Source: CAD feature listing. Evaluate the final solid. Frame: model axes, mm. Face numbers are marked on the shaded views. Give positions to 0.01 mm unless a question says otherwise; leave off trailing zeros. Loops run counter-clockwise (first coordinate to the right, second up) from the corner with the lowest first, then second, coordinate; pieces in that order, holes last. Notation, with made-up numbers: M -28,-6 L -12,-6 A18 cw -12,27 Z; hole C 35,62.25 d2. An arc over 180 degrees is marked long. Write item = value, one per line.
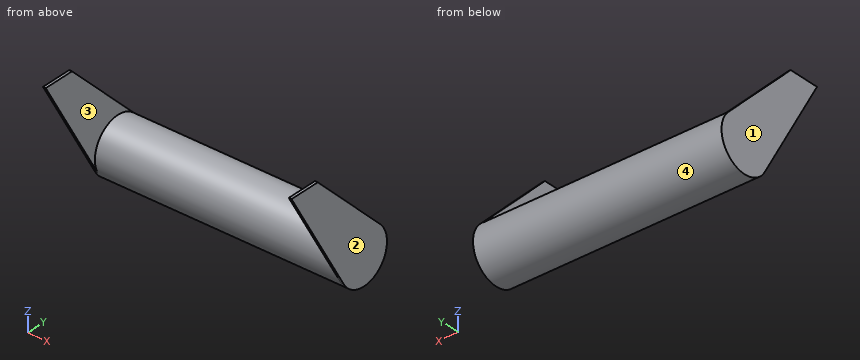
from build123d import *

# Parameters (mm, degrees)
SKETCH1_R           = 10
SKETCH1_R_2         = 9
BOSS_EXTRUDE1_DEPTH = 45
SKETCH2_R           = 10
SKETCH2_R_2         = 9
BOSS_EXTRUDE2_DEPTH = 1


with BuildPart() as part:
    # Sketch1 → Boss-Extrude1 (new, symmetric)
    with BuildSketch(Plane(origin=(0, 0, 0), x_dir=(0, 0, -1), z_dir=(1, 0, 0))):
        with Locations(Location((0, 0, 0), (0, 0, 180))):
            Circle(SKETCH1_R)
        with Locations(Location((0, 0, 0), (0, 0, 180))):
            Circle(SKETCH1_R_2, mode=Mode.SUBTRACT)
    extrude(amount=BOSS_EXTRUDE1_DEPTH, both=True)

    # Sketch2 → Boss-Extrude2 (add)
    # profile 1 of 3: a face of its own
    with BuildSketch(Plane(origin=(45, 0, 0), x_dir=(0, 0, -1), z_dir=(1, 0, 0))):
        with BuildLine():
            ThreePointArc((5, -8.660254038), (-7.933533403, -6.08761429), (-7.071067812, 7.071067812))
            Line((-7.071067812, 7.071067812), (-34, -19.857864376))
            Line((-34, -19.857864376), (-34, -31.176914536))
            Line((-34, -31.176914536), (5, -8.660254038))
        make_face()
    # profile 2 of 3: a face of its own
    with BuildSketch(Plane(origin=(45, 0, 0), x_dir=(0, 0, -1), z_dir=(1, 0, 0))):
        with Locations(Location((0, 0, 0), (0, 0, 135))):
            Circle(SKETCH2_R)
        with Locations(Location((0, 0, 0), (0, 0, 180))):
            Circle(SKETCH2_R_2, mode=Mode.SUBTRACT)
    # profile 3 of 3: a face of its own
    with BuildSketch(Plane(origin=(45, 0, 0), x_dir=(0, 0, -1), z_dir=(1, 0, 0))):
        with Locations(Location((0, 0, 0), (0, 0, 180))):
            Circle(SKETCH2_R_2)
    boss_extrude2 = extrude(amount=-BOSS_EXTRUDE2_DEPTH)

    # Mirror1: Boss-Extrude2 across plane
    add(boss_extrude2.mirror(Plane(origin=(0, 0, 0), x_dir=(0, 0, 1), z_dir=(1, 0, 0))))


solid = part.part
1. Cut plane C-C, the plane y = -5. Return the cut outline in (x, z), then the cut area to 3 significant figures.
Derived:
outline = M -45,-8.66 L 45,-8.66 L 45,19.14 L 44,19.14 L 44,8.66 L -44,8.66 L -44,19.14 L -45,19.14 Z; hole M -44,-7.48 L 44,-7.48 L 44,7.48 L -44,7.48 Z
area = 263 mm²
2. Pull-direction query (X, two-part tool) for the marked faces 1, 2, 3 and 4; classes: +X half, -X half, draft (parallel to the pull), parting line (faces both ways), or undercut.
Derived:
face_1 = -X half
face_2 = +X half
face_3 = undercut
face_4 = undercut
3. First-contact query: pin 1 Ø3 at (x, y) = (34, 2.5) entering from +Z; pin 2 Ø2 at (y, z) = (-13.5, -2.5) entering from +X. Flat tips, straight axial feed; report the tip coordinate or a pass-through.
Derived:
pin_1 = 9.95
pin_2 = through
4. Material intervals for probe 1 along Y at (x, z) = (8, 0); probe 2 along X at (y, z) = (-20.5, 23.5); probe 3 along Z at (x, y) = (-40, 5.5), sorted ascending. Write a range as from..to.
Derived:
probe_1 = -10..-9, 9..10
probe_2 = -45..-44, 44..45
probe_3 = -8.35..-7.12, 7.12..8.35
5. Cut plane D-D, the plane z = 21. Return the cut outline in (x, y), then the cut area to 3 significant figures.
Derived:
outline = M -45,-23.67 L -44,-23.67 L -44,-6.86 L -45,-6.86 Z; M 44,-23.67 L 45,-23.67 L 45,-6.86 L 44,-6.86 Z
area = 33.6 mm²
6. Cut plane B-B, the plane z = 8. Return the cut outline in (x, y), then the cut area to 3 significant figures.
Derived:
outline = M -45,-16.17 L -44,-16.17 L -44,-6 L 44,-6 L 44,-16.17 L 45,-16.17 L 45,6.14 L 44,6.14 L 44,6 L -44,6 L -44,6.14 L -45,6.14 Z; hole M -44,-4.12 L 44,-4.12 L 44,4.12 L -44,4.12 Z
area = 375 mm²
7. Cut plane A-A, the plane y = -21. Return the cut outline in (x, z).
Derived:
outline = M -45,16.37 L -44,16.37 L -44,34 L -45,34 Z; M 44,16.37 L 45,16.37 L 45,34 L 44,34 Z
